Can you work these out from the model? Positions are in its coordinate system, mm. Round coordinates to 2 decimals unless told otherwise and drop trailing zeros. Order: outer loops, then holes, each group sorted by start corner. A loop starts at its lowest first (then second) coordinate and runs counter-clockwise, first axis right, second up. Notation, with made-up numbers: (-18.75, -15) - (-6.75, -15) arc R28 cw to (-6.75, 10) - close; hole circle Ø5 at (24.5, -38). An arc over 180 degrees is marked (long way). Write item = value, one per line.
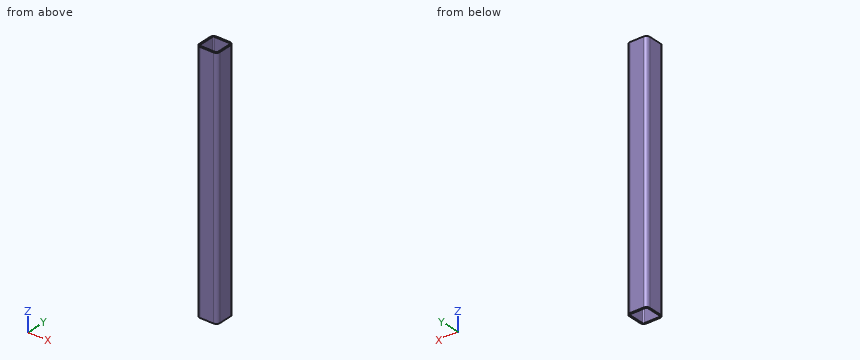
from build123d import *

# Parameters (mm, degrees)
SKETCH1_W           = 40
SKETCH1_H           = 40
SKETCH1_W_2         = 34
SKETCH1_H_2         = 34
BOSS_EXTRUDE1_DEPTH = 479.48
FILLET1_R           = 2
FILLET2_R           = 7


with BuildPart() as part:
    # Sketch1 → Boss-Extrude1 (new body)
    with BuildSketch(Plane.XY):
        Rectangle(SKETCH1_W, SKETCH1_H)
        Rectangle(SKETCH1_W_2, SKETCH1_H_2, mode=Mode.SUBTRACT)
    extrude(amount=BOSS_EXTRUDE1_DEPTH)

    # Fillet1
    fillet1_edges = [part.edges().sort_by_distance(p)[0] for p in [
        (17, -17, 239.74),
        (17, 17, 239.74),
        (-17, 17, 239.74),
        (-17, -17, 239.74),
    ]]
    fillet(fillet1_edges, radius=FILLET1_R)

    # Fillet2
    fillet2_edges = [part.edges().sort_by_distance(p)[0] for p in [
        (20, -20, 239.74),
        (-20, -20, 239.74),
        (-20, 20, 239.74),
        (20, 20, 239.74),
    ]]
    fillet(fillet2_edges, radius=FILLET2_R)


solid = part.part
(1) If I drill on line 1 (Y direction, x = -7, z = 168); line 2 (X direction, y = 16.5, z = 265), over which ranges is the centre line in solid material (lowest first)? Write a range as from..to.
Computed:
line_1 = -20..-17, 17..20
line_2 = -19.06..-16.32, 16.32..19.06
(2) If we section it at A-A (y = -1): Write out the boundary of the cut face in (x, z), plus the area to 3 significant figures.
Computed:
outline = (-20, 0) - (-17, 0) - (-17, 479.48) - (-20, 479.48) - close; (17, 0) - (20, 0) - (20, 479.48) - (17, 479.48) - close
area = 2,880 mm^2
(3) Will these pins go through, and if not, where does the flat tip stop? P1, Ø10, axis at y = 15, z = 350.5, coming from the +X side; P2, Ø1, axis at x = 15, z = 50, coming from the +Y side.
Computed:
P1 = 20
P2 = 19.84
(4) If we section it at C-C (z = 120): Write out the boundary of the cut face in (x, y).
Computed:
outline = (-20, -13) arc R7 ccw to (-13, -20) - (13, -20) arc R7 ccw to (20, -13) - (20, 13) arc R7 ccw to (13, 20) - (-13, 20) arc R7 ccw to (-20, 13) - close; hole (-17, -15) arc R2 ccw to (-15, -17) - (15, -17) arc R2 ccw to (17, -15) - (17, 15) arc R2 ccw to (15, 17) - (-15, 17) arc R2 ccw to (-17, 15) - close
